Verification items for the finished model (mm, model axes). Face numbers are marked on the shaded views. Round coordinates to 2 decimals unless told otherwise and drop trailing zeros. Order: outer loops, then holes, each group sorted by start corner. A loop starts at its lowest first (then second) coordinate and runs counter-clockwise, first axis right, second up. Notation, with made-up numbers: (54, -25) -> (73, -25) arc R19 cw to (73, -7) -> close; hole circle Ø2 at (32, 9). An arc over 180 degrees is marked (long way). Put each result on its own line as item: value.
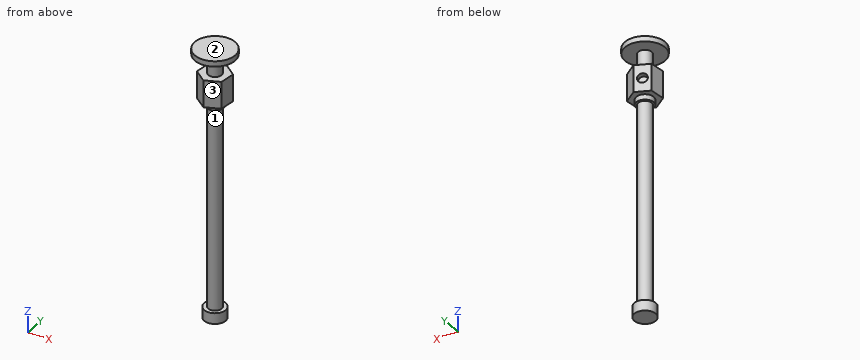
from build123d import *

# Parameters (mm, degrees)
SKETCH2_R           = 2.5
BOSS_EXTRUDE1_DEPTH = 100
SKETCH3_R           = 4
BOSS_EXTRUDE2_DEPTH = 4
SKETCH4_R           = 7.5
BOSS_EXTRUDE3_DEPTH = 2
BOSS_EXTRUDE4_DEPTH = 10
SKETCH6_R           = 3.25
BOSS_EXTRUDE5_DEPTH = 2
SKETCH7_R           = 1.75
CUT_EXTRUDE1_DEPTH  = 2


with BuildPart() as part:
    # Sketch2 → Boss-Extrude1 (new body)
    with BuildSketch(Plane.XY):
        with Locations((20.609067119, -9.310698144)):
            Circle(SKETCH2_R)
    extrude(amount=BOSS_EXTRUDE1_DEPTH)

    # Sketch3 → Boss-Extrude2 (add)
    with BuildSketch(Plane(origin=(0, 0, 0), x_dir=(-1, 0, 0), z_dir=(0, 0, -1))):
        with Locations((-20.609067119, -9.310698144)):
            Circle(SKETCH3_R)
    extrude(amount=-BOSS_EXTRUDE2_DEPTH)

    # Sketch4 → Boss-Extrude3 (add)
    with BuildSketch(Plane.XY.offset(100)):
        with Locations((20.609067119, -9.310698144)):
            Circle(SKETCH4_R)
    extrude(amount=-BOSS_EXTRUDE3_DEPTH)

    # Sketch5 → Boss-Extrude4 (add)
    with BuildSketch(Plane(origin=(0, 0, 91), x_dir=(-1, 0, 0), z_dir=(0, 0, -1))):
        Polygon((-16.079485871, -5.730722299), (-21.444626522, -3.597977792), (-25.97420777, -7.177953637), (-25.138648367, -12.890673989), (-19.773507717, -15.023418496), (-15.243926469, -11.443442651), align=None)
    extrude(amount=BOSS_EXTRUDE4_DEPTH)

    # Sketch6 → Boss-Extrude5 (add)
    with BuildSketch(Plane(origin=(0, 0, 81), x_dir=(-1, 0, 0), z_dir=(0, 0, -1))):
        with Locations((-20.609067119, -9.310698144)):
            Circle(SKETCH6_R)
    extrude(amount=BOSS_EXTRUDE5_DEPTH)

    # Sketch7 → Cut-Extrude1 (cut)
    with BuildSketch(Plane(origin=(4.161383334, -10.468392636, 0), x_dir=(0.9292696196810543, 0.3694021845331033, 0), z_dir=(-0.3694021845331033, 0.9292696196810543, 0))):
        with Locations(Location((15.71198773, -86, 0), (0, 0, 180))):
            Circle(SKETCH7_R)
    extrude(amount=-CUT_EXTRUDE1_DEPTH, mode=Mode.SUBTRACT)


solid = part.part
Item 1: Release check for a two-part mould opening along Z. For the marked faces 1, 2 and 3 record: +Z half, -Z half, draft (parallel to the pull), parting line (faces both ways), or undercut.
Check sheet entries:
face 1: undercut
face 2: +Z half
face 3: draft
Item 2: Material ranges on L1, parallel to Z at x = 20.5, y = -13.25; L2, parallel to Z at x = 19.5, y = -14.75; L3, parallel to Z at x = 14.25, y = -8.75, recorded low to high. Write a range as [from, to].
Check sheet entries:
L1: z = [0, 4], [81, 91], [98, 100]
L2: z = [81, 91], [98, 100]
L3: z = [98, 100]
Item 3: Section check A-A on z = 39. Record the boundary of the cut face in (x, y).
Check sheet entries:
outline: circle Ø5 at (20.61, -9.31)
Item 4: Gauge pin test, flat ends, axial feed: pin 1 Ø1.5 at (y, z) = (-12, 11.5) entering from +X; pin 2 Ø1 at (x, y) = (25.5, -6.5) entering from -Z; pin 3 Ø4 at (x, z) = (23, 40.5) entering from +Y. Record the tip position at first contact, or that the pin passes through.
Check sheet entries:
pin 1: stops at x = 22.19
pin 2: stops at z = 81
pin 3: stops at y = -6.84
